Answer from the drawing. Dimensions are ordinates in mm from the lowest x, y and z of the part. Coordinates: 2 decimals unless noted, no trailing zeros. Order: outer loops, then holes, each group sorted by start corner. A loop starts at its lowest first (then second) coordinate and runs counter-clockwise, first axis right, second up. Notation, with made-up numbers: (14.25, -33.5) - (53.25, -33.5) arc R10 cw to (53.25, -15.5) - close; hole circle Ø1 at (54.25, 2). An arc over 180 degrees is marked (long way). Answer as a JSON object with one key per item and string values. Group by question number.
1) Section D-D (z = 854.5) is taken. Give the vertices of the cut face in (x, y) (1 decimal).
2) This flat-tipped pin is pushed along its axis until it touches: P1, Ø1.5, axis at y = 6.5, z = 603, coming from the +X side. Where does it stop, or does it pass through?
3) Section C-C (y = 3.25) is taken. Count the separate pieces of the cut face and the enclosed holes in it, plus the area to 3 significant figures.
4) Section B-B (z = 500) is taken. Give the vertices of the cut face in (x, y), plus the area to 3 significant figures.
5) Find the intervals of material crossed by line 1 along X through (y, z) = (5.25, 510); line 2 along X through (y, z) = (5.5, 500); line 3 along Z through (x, y) = (704, 0.5), in increasing order.
6) Section A-A (x = 500) is taken. Give the vertices of the cut face in (y, z).
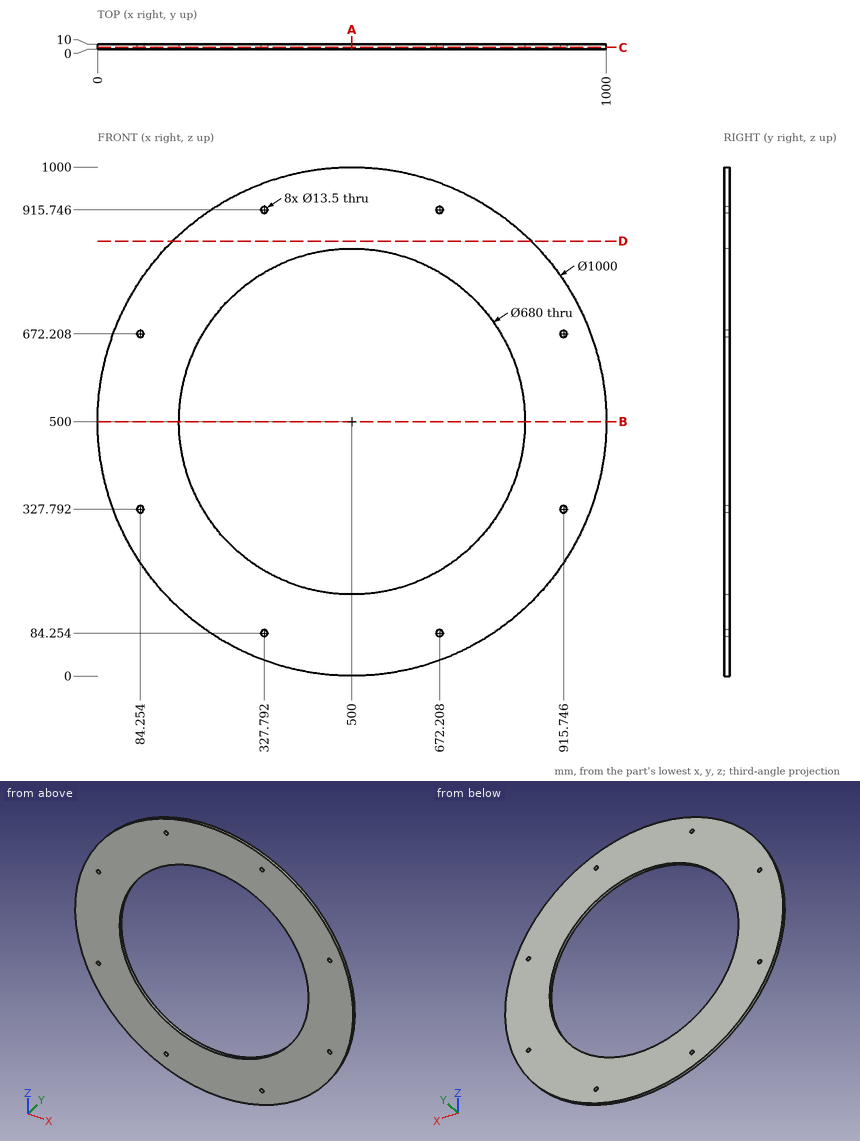
Report:
{
 "1": {"outline": "(147.4, 0) - (852.6, 0) - (852.6, 10) - (147.4, 10) - close"},
 "2": {"P1": "stops at x = 989.43"},
 "3": {"separate pieces": "1", "enclosed holes": "9", "area": "421,000 mm²"},
 "4": {"outline": "(0, 0) - (160, 0) - (160, 10) - (0, 10) - close; (840, 0) - (1000, 0) - (1000, 10) - (840, 10) - close", "area": "3,200 mm²"},
 "5": {"line 1": "x = 0.1 to 160.15, 839.85 to 999.9", "line 2": "x = 0 to 160, 840 to 1000", "line 3": "z = 43.51 to 228, 772 to 956.49"},
 "6": {"outline": "(0, 0) - (10, 0) - (10, 160) - (0, 160) - close; (0, 840) - (10, 840) - (10, 1000) - (0, 1000) - close"}
}
